from build123d import *

# Parameters (mm, degrees)
SKETCH_1_W      = 18.5
SKETCH_1_H      = 55
EXTRUDE_1_DEPTH = 7
SKETCH_2_R      = 3.5
EXTRUDE_2_DEPTH = 55


with BuildPart() as part:
    # 草图1 → 凸台-拉伸1 (new body)
    with BuildSketch(Plane.XY):
        with Locations((9.25, 27.5)):
            Rectangle(SKETCH_1_W, SKETCH_1_H)
    extrude(amount=EXTRUDE_1_DEPTH)

    # 草图2 → 凸台-拉伸2 (add)
    with BuildSketch(Plane(origin=(0, 55, 0), x_dir=(1, 0, 0), z_dir=(0, 1, 0))):
        with Locations((20, -5)):
            Circle(SKETCH_2_R)
    extrude(amount=-EXTRUDE_2_DEPTH)


solid = part.part
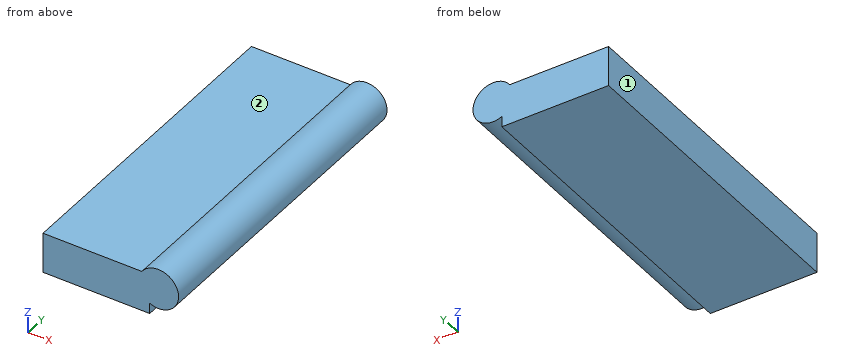
The model under review builds one solid part; all positions refer to its coordinate system, in mm. Face numbers are marked on the shaded views. A direction names the side the tool comes from. Coordinates: 2 decimals unless noted, no trailing zeros. Loops run counter-clockwise (first coordinate to the right, second up) from the corner with the lowest first, then second, coordinate; pieces in that order, holes last. Notation, with made-up numbers: M 42,16.5 L 51,16.5 A14 cw 51,26.5 Z; hole C 55,-16 d6. An arc over 180 degrees is marked long. Put each result on its own line as item: value. Start each with the question number.
Q1. Add section C-C (z = 1). Write out the cut boundary in (x, y), and give its area (3 significant figures).
Q2. Wall thickness on line 1 (Z direction, x = 1.25, y = 49); line 2 (X direction, y = 34, z = 5.25); line 3 (X direction, y = 51, z = 1.25): over which ranges is each line inside the solid? List them lowest first.
Q3. Clearance check with flat-ended pins moving along their axes: pin 1 (8.5 mm diameter, centred on x = 11, y = 25.5, fed in from +Z); pin 2 (5 mm diameter, centred on y = 18.5, z = 2, fed in from +X). State where each tip first meets the part, or that it passes through.
Q4. Add section B-B (x = 20). Write out the cut boundary in (y, z).
Q5. Add section A-A (y = 18.5). Write out the cut boundary in (x, z).
Q6. For the marked faces 1 and 2, list the 3-axis set-ups (+Z, -Z, +X, -X, +Y, -Y) from which the entire face can be reached by the end or side of a thin tool; tool diameter is ignored.
Answers:
1. outline: M 0,0 L 18.5,0 L 18.5,55 L 0,55 Z
1. area: 1,020 mm^2
2. line 1: z = 0 to 7
2. line 2: x = 0 to 23.49
2. line 3: x = 0 to 18.5
3. pin 1: stops at z = 7
3. pin 2: stops at x = 23.46
4. outline: M 0,1.5 L 55,1.5 L 55,8.5 L 0,8.5 Z
5. outline: M 0,0 L 18.5,0 L 18.5,1.84 A3.5 ccw long 17.13,7 L 0,7 Z
6. face 1: +Z, -Z, -X, +Y, -Y
6. face 2: +Z, -X, +Y, -Y
